Can you work these out from the model? Positions are in its coordinate system, mm. A direction names the side the tool comes from. Give positions to 0.01 mm unless a question says otherwise; leave off trailing zeros. Loops run counter-clockwise (first coordinate to the right, second up) from the corner with the lowest first, then second, coordinate; pieces in that order, holes last. Notation, with made-up numbers: (78, 2) - (117, 2) arc R26 cw to (117, 24) - close; hole circle Ø5 at (60.25, 8). An arc over 180 degrees is marked (long way). Write item = value, one per line.
from build123d import *

# Parameters (mm, degrees)
SKETCH1_R             = 50
SKETCH1_R_2           = 40
BOSS_EXTRUDE1_DEPTH   = 741
SKETCH2_R             = 61.681035311
SKETCH2_R_2           = 47.5
CUT_EXTRUDE1_DEPTH    = 45
CHAMFER1_SIZE         = 1
CHAMFER2_SIZE         = 1
SKETCH10_R            = 42.5
CUT_EXTRUDE9_DEPTH    = 10
SKETCH11_R            = 41.5
CUT_EXTRUDE10_DEPTH   = 50
M6_TAPPED_HOLE1_D     = 5
M6_TAPPED_HOLE1_DEPTH = 15
M6_TAPPED_HOLE1_TIP   = 1.502151548


with BuildPart() as part:
    # Sketch1 → Boss-Extrude1 (new body)
    with BuildSketch(Plane.XY):
        Circle(SKETCH1_R)
        Circle(SKETCH1_R_2, mode=Mode.SUBTRACT)
    extrude(amount=BOSS_EXTRUDE1_DEPTH)

    # Sketch2 → Cut-Extrude1 (cut)
    with BuildSketch(Plane(origin=(0, 0, 0), x_dir=(-1, 0, 0), z_dir=(0, 0, -1))):
        Circle(SKETCH2_R)
        Circle(SKETCH2_R_2, mode=Mode.SUBTRACT)
    extrude(amount=-CUT_EXTRUDE1_DEPTH, mode=Mode.SUBTRACT)

    # Chamfer1
    chamfer1_edges = [part.edges().sort_by_distance(p)[0] for p in [
        (47.5, 0, 0),
    ]]
    chamfer(chamfer1_edges, length=CHAMFER1_SIZE)

    # Chamfer2
    chamfer2_edges = [part.edges().sort_by_distance(p)[0] for p in [
        (-50, 0, 741),
    ]]
    chamfer(chamfer2_edges, length=CHAMFER2_SIZE)

    # Sketch10 → Cut-Extrude9 (cut)
    with BuildSketch(Plane.XY.offset(741)):
        Circle(SKETCH10_R)
    extrude(amount=-CUT_EXTRUDE9_DEPTH, mode=Mode.SUBTRACT)

    # Sketch11 → Cut-Extrude10 (cut)
    with BuildSketch(Plane.XY.offset(731)):
        Circle(SKETCH11_R)
    extrude(amount=-CUT_EXTRUDE10_DEPTH, mode=Mode.SUBTRACT)

    # M6 Tapped Hole1
    with Locations(Plane.XZ.offset(50)):
        with Locations((0, 728)):
            Hole(M6_TAPPED_HOLE1_D / 2, depth=M6_TAPPED_HOLE1_DEPTH)
            with Locations((0, 0, -(M6_TAPPED_HOLE1_DEPTH + M6_TAPPED_HOLE1_TIP / 2))):  # 118° drill point
                Cone(0, M6_TAPPED_HOLE1_D / 2, M6_TAPPED_HOLE1_TIP, mode=Mode.SUBTRACT)


solid = part.part
Q1. We'd pull the mould along X, two halves only. Please class faces 4 (the cylindrical face through (-8.67, -39.05, 335.73)), 5 (the cylindrical face through (47.69, 15.02, 387.64)), 6 (the flat face through (9, -41, 731)), 7 (the flat face through (-44.2, -18.3, 45)): released by +X, released by -X, zero draft, split by the parting line, or undercut.
Output:
face_4 = undercut
face_5 = split by the parting line
face_6 = undercut
face_7 = zero draft
Q2. Which directions (+Z, -Z, +X, -X, +Y, -Y) give clear straight access to the entire face, cutting with the end or side of a thin tool? Please do faces 1 (the cylindrical face through (10.3, -46.37, 22.69)), 2 (the flat face through (-15, 40, 741)), 3 (the cylindrical face through (-33.727, -25.861, 736.07)).
Output:
face_1 = -Z
face_2 = +Z, +X, -X, +Y, -Y
face_3 = +Z
Q3. Imagine slicing it at A-A, the plane y = 0. Write out the boundary of the cut face in (x, z).
Output:
outline = (-50, 45) - (-47.5, 45) - (-47.5, 1) - (-46.5, 0) - (-40, 0) - (-40, 681) - (-41.5, 681) - (-41.5, 731) - (-42.5, 731) - (-42.5, 741) - (-49, 741) - (-50, 740) - close; (40, 0) - (46.5, 0) - (47.5, 1) - (47.5, 45) - (50, 45) - (50, 740) - (49, 741) - (42.5, 741) - (42.5, 731) - (41.5, 731) - (41.5, 681) - (40, 681) - close
Q4. I need wall thicknesses on L1, parallel to Y at x = 0, z = 358; L2, parallel to Z at x = 0, y = -43.25; L3, parallel to Y at x = 0, z = 694. Which ranges of each line are inside material? Lowest first, please.
Output:
L1 = -50 to -40, 40 to 50
L2 = 0 to 725.5, 730.5 to 741
L3 = -50 to -41.5, 41.5 to 50
Q5. Imagine slicing it at B-B, the plane z = 334. Write out the boundary of the cut face in (x, y).
Output:
outline = circle Ø100 at (0, 0); hole circle Ø80 at (0, 0)
Q6. For pin 1 (8 mm diameter, centred on x = 0, z = 728, fed in from +Y); pin 2 (8 mm diameter, centred on y = -13, z = 537.5, fed in from -X); pin 3 (8 mm diameter, centred on y = -20.5, z = 294, fed in from -X), each with a flat end and sliding along its axis, tell me the tip position at first contact or that it passes through.
Output:
pin_1 = 50
pin_2 = -49.18
pin_3 = -47.2
